Geometry check sheet. Reference: drawing and pictorial views, mm from the part's lowest x, y, z. Give positions to 0.01 mm unless a question says otherwise; leave off trailing zeros. Write each loop counter-clockwise with the first axis right and the second up, starting at its lowest first coordinate (ties: lowest second). Pieces come first, ordered by that corner, then holes.
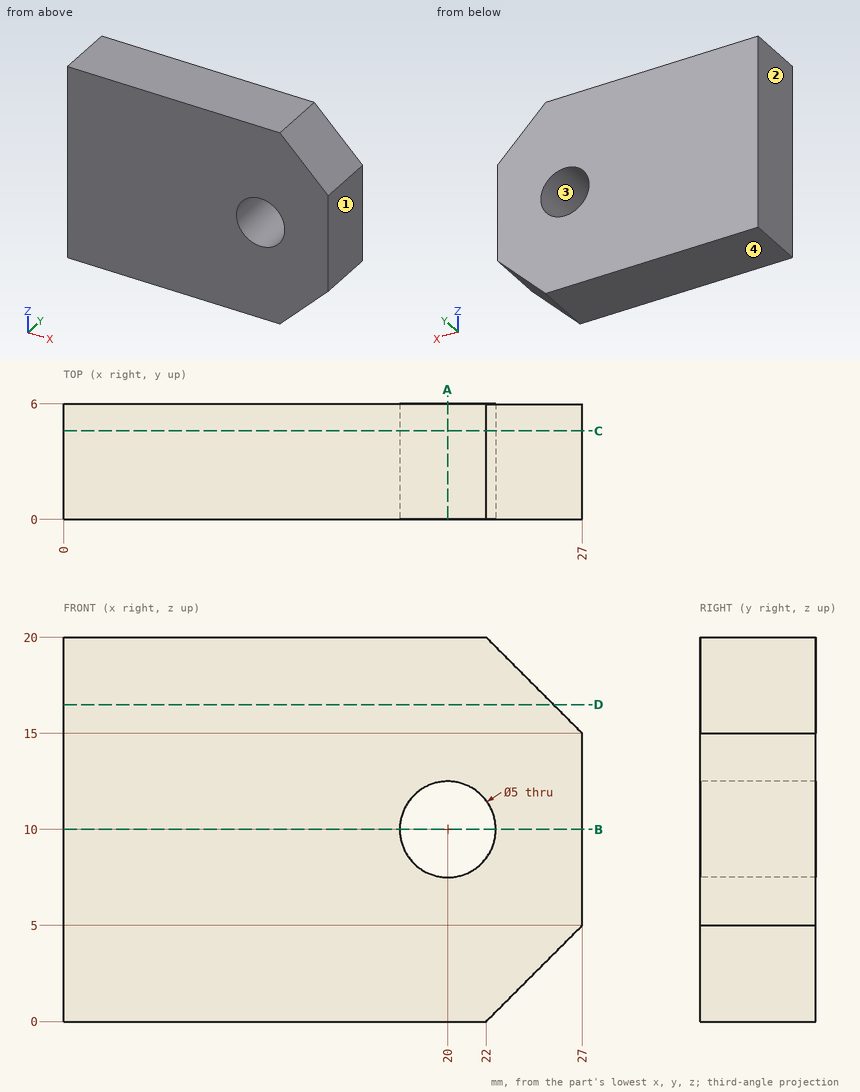
Item 1: Scan lines: line 1 along X through (y, z) = (3.15, 10); line 2 along Z through (x, y) = (20, 1.75); line 3 along Z through (x, y) = (20.5, 4.35). Record each from-to range of solid material in increasing order.
Answer key:
line 1: x = 0 to 17.5, 22.5 to 27
line 2: z = 0 to 7.5, 12.5 to 20
line 3: z = 0 to 7.55, 12.45 to 20
Item 2: Sectioned sample at C-C on y = 4.6. Record the cut outline in (x, z).
Answer key:
outline: (0, 0) - (22, 0) - (27, 5) - (27, 15) - (22, 20) - (0, 20) - close; hole circle Ø5 at (20, 10)
Item 3: Sectioned sample at A-A on x = 20. Record the cut outline in (y, z).
Answer key:
outline: (0, 0) - (6, 0) - (6, 7.5) - (0, 7.5) - close; (0, 12.5) - (6, 12.5) - (6, 20) - (0, 20) - close
Item 4: Sectioned sample at B-B on z = 10. Record the cut outline in (x, y).
Answer key:
outline: (0, 0) - (17.5, 0) - (17.5, 6) - (0, 6) - close; (22.5, 0) - (27, 0) - (27, 6) - (22.5, 6) - close
Item 5: Release check for a two-part mould opening along X. For the marked faces 1, 2, 3 and 4 record: released by +X, released by -X, zero draft, split by the parting line, or undercut.
Answer key:
face 1: released by +X
face 2: released by -X
face 3: undercut
face 4: zero draft
Item 6: Sectioned sample at D-D on z = 16.5. Record the cut outline in (x, y).
Answer key:
outline: (0, 0) - (25.5, 0) - (25.5, 6) - (0, 6) - close
Item 7: Depth check by flat-ended pin: pin 1 (3 mm diameter, centred on x = 20, z = 10, fed in from -Y). Enter the tip coordinate at first touch or a pass-through.
Answer key:
pin 1: passes through
